Could you check a few things on this model? Use its own coordinates, in mm. A direction names the side the tool comes from. Give positions to 0.01 mm unless a question says otherwise; leave off trailing zeros. Loops run counter-clockwise (first coordinate to the right, second up) from the corner with the lowest first, then second, coordinate; pieces in that order, holes last.
1. I need wall thicknesses on line 1 along Z through (x, y) = (41, 6); line 2 along Z through (x, y) = (41, 11); line 3 along X through (y, z) = (9.75, 31). Which ranges of each line are inside material? Lowest first, please.
2. Imagine slicing it at B-B (x = 0). List the corners of the cut face in (y, z) for me, plus the area to 4 significant figures.
3. For P1, Ø5.5, axis at x = -41, z = -26, coming from the -Y side; P2, Ø10.5, axis at x = 41, z = -26, coming from the +Y side; P3, Ø12.5, axis at x = -41, z = -26, coming from the -Y side; P4, Ø10, axis at x = -37.5, z = -12, coming from the +Y side, each with a flat end and sliding along its axis, tell me the tip position at first contact or that it passes through.
4. Imagine slicing it at D-D (y = -1.25). List the corners of the cut face in (x, z) for me, plus the area to 3 significant figures.
5. Thinking about a two-plate mould opening in Z: for faces 4 (the flat face through (50, 7, 1)), 5 (the flat face through (-47, 7, 48)), 6 (the cylindrical face through (43.619, 3.993, -23.992)), which applies, +Z half, -Z half, draft (parallel to the pull), parting line (faces both ways), or undercut?
6. Imagine slicing it at C-C (y = 11.5). Count the separate pieces of the cut face and the enclosed holes in it, plus the area to 3 significant figures.
7. Imagine slicing it at A-A (z = 0). List the corners of the cut face in (x, y) for me, plus the area to 4 significant figures.
8. For faces 1 (the flat face through (41, 8.1, 30)), 2 (the cylindrical face through (10.81, -1.23, -34.34)), 3 (the flat face through (-50, 7, 1)), which set-ups out of +Z, -Z, +X, -X, +Y, -Y let a thin tool reach every point of the face, with its end or its side?
```python
from build123d import *

# Parameters (mm, degrees)
SKETCH_1_W                   = 100
SKETCH_1_H                   = 100
EXTRUDE_1_DEPTH              = 14.5
SKETCH_3_R                   = 36
SKETCH_3_R_2                 = 33
EXTRUDE_2_DEPTH              = 3
SKETCH_4_R                   = 33
CUT_EXTRUDE_1_DEPTH          = 73.182061483
CHAMFER_1_SIZE               = 5
CHAMFER_2_SIZE               = 0.5
SKETCH_10_R                  = 40
CUT_EXTRUDE_3_DEPTH          = 8
HOLE_WIZARD_M6_1_D           = 5
HOLE_WIZARD_M6_1_DEPTH       = 15
HOLE_WIZARD_M6_1_TIP         = 1.502151548
HOLE_WIZARD_M6_2_D           = 6.6
HOLE_WIZARD_M6_2_CBORE_D     = 11
HOLE_WIZARD_M6_2_CBORE_DEPTH = 6.4
CHAMFER_3_SIZE               = 0.5


with BuildPart() as part:
    # 草图1 → 凸台-拉伸1 (new body)
    with BuildSketch(Plane(origin=(0, 0, 0), x_dir=(1, 0, 0), z_dir=(0, 1, 0))):
        Rectangle(SKETCH_1_W, SKETCH_1_H)
    extrude(amount=EXTRUDE_1_DEPTH)

    # 草图3 → 凸台-拉伸2 (add)
    with BuildSketch(Plane.XZ):
        with Locations(Location((0, 0, 0), (0, 0, 270))):
            Circle(SKETCH_3_R)
        with Locations(Location((0, 0, 0), (0, 0, 270))):
            Circle(SKETCH_3_R_2, mode=Mode.SUBTRACT)
    extrude(amount=EXTRUDE_2_DEPTH)

    # 草图4 → 切除-拉伸1 (cut, through all)
    with BuildSketch(Plane.XZ):
        with Locations(Location((0, 0, 0), (0, 0, 270))):
            Circle(SKETCH_4_R)
    extrude(amount=-CUT_EXTRUDE_1_DEPTH, mode=Mode.SUBTRACT)

    # 倒角1
    chamfer_1_edges = [part.edges().sort_by_distance(p)[0] for p in [
        (50, 7.25, 50),
        (-50, 7.25, 50),
        (-50, 7.25, -50),
        (50, 7.25, -50),
    ]]
    chamfer(chamfer_1_edges, length=CHAMFER_1_SIZE)

    # 倒角2
    chamfer_2_edges = [part.edges().sort_by_distance(p)[0] for p in [
        (0, -3, 36),
    ]]
    chamfer(chamfer_2_edges, length=CHAMFER_2_SIZE)

    # 草图10 → 切除-拉伸3 (cut)
    with BuildSketch(Plane(origin=(0, 14.5, 0), x_dir=(1, 0, 0), z_dir=(0, 1, 0))):
        with Locations(Location((0, 0, 0), (0, 0, 270))):
            Circle(SKETCH_10_R)
    extrude(amount=-CUT_EXTRUDE_3_DEPTH, mode=Mode.SUBTRACT)

    # Hole Wizard M6 _1
    with Locations(Plane(origin=(0, 14.5, 0), x_dir=(1, 0, 0), z_dir=(0, 1, 0))):
        with Locations((-35.355, 35.355), (0, 0), (35.355, 35.355), (-35.355, -35.355), (35.355, -35.355)):
            Hole(HOLE_WIZARD_M6_1_D / 2, depth=HOLE_WIZARD_M6_1_DEPTH)
            with Locations((0, 0, -(HOLE_WIZARD_M6_1_DEPTH + HOLE_WIZARD_M6_1_TIP / 2))):  # 118° drill point
                Cone(0, HOLE_WIZARD_M6_1_D / 2, HOLE_WIZARD_M6_1_TIP, mode=Mode.SUBTRACT)

    # M6 六角凹头螺钉的柱形沉头孔2 (through all)
    with Locations(Plane(origin=(0, 14.5, 0), x_dir=(1, 0, 0), z_dir=(0, 1, 0))):
        with Locations((-41, 26), (0, 0), (41, -26), (41, 26), (-41, -26)):
            CounterBoreHole(HOLE_WIZARD_M6_2_D / 2, HOLE_WIZARD_M6_2_CBORE_D / 2, HOLE_WIZARD_M6_2_CBORE_DEPTH)

    # 倒角3
    chamfer_3_edges = [part.edges().sort_by_distance(p)[0] for p in [
        (0, 14.5, -40),
    ]]
    chamfer(chamfer_3_edges, length=CHAMFER_3_SIZE)


solid = part.part
```
Derived:
1. line 1: z = -50 to -29.3, -22.7 to 22.7, 29.3 to 50
1. line 2: z = -50 to -31.5, -20.5 to 20.5, 31.5 to 50
1. line 3: x = -50 to -43.29, -38.71 to -25.28, 25.28 to 38.71, 43.29 to 50
2. outline: (-3, -35.5) - (-2.5, -36) - (0, -36) - (0, -50) - (14.5, -50) - (14.5, -40.5) - (14, -40) - (6.5, -40) - (6.5, -33) - (-3, -33) - close; (-3, 33) - (6.5, 33) - (6.5, 40) - (14, 40) - (14.5, 40.5) - (14.5, 50) - (0, 50) - (0, 36) - (-2.5, 36) - (-3, 35.5) - close
2. area: 398.5 mm2
3. P1: passes through
3. P2: stops at y = 8.1
3. P3: stops at y = 0
3. P4: stops at y = 14.5
4. outline: circle Ø72 at (0, 0); hole circle Ø66 at (0, 0)
4. area: 650 mm2
5. face 4: draft
5. face 5: +Z half
5. face 6: undercut
6. separate pieces: 1
6. enclosed holes: 9
6. area: 4,460 mm2
7. outline: (-50, 0) - (-36, 0) - (-36, -2.5) - (-35.5, -3) - (-33, -3) - (-33, 6.5) - (-40, 6.5) - (-40, 14) - (-40.5, 14.5) - (-50, 14.5) - close; (33, -3) - (35.5, -3) - (36, -2.5) - (36, 0) - (50, 0) - (50, 14.5) - (40.5, 14.5) - (40, 14) - (40, 6.5) - (33, 6.5) - close
7. area: 398.5 mm2
8. face 1: +Y
8. face 2: -Y
8. face 3: +Z, -Z, -X, +Y, -Y
